Can you work these out from the model? Positions are in its coordinate system, mm. A direction names the side the tool comes from. Coordinates: 2 decimals unless noted, no trailing zeros. Loops run counter-clockwise (first coordinate to the right, second up) from the corner with the lowest first, then second, coordinate; pieces in that order, holes last. Notation, with made-up numbers: (64, 5) -> (83, 5) arc R18 ccw to (83, 14) -> close; hole circle Ø8 at (-15.5, -38). An arc over 180 degrees is marked (long way). Use one line per item in the form item = value. Start each with the question number.
(1) I'm going to push flat-ended pins straight in: pin 1 (2.5 mm diameter, centred on y = 11.5, z = 9.5, fed in from +X); pin 2 (3.5 mm diameter, centred on y = 4.45, z = 4, fed in from +X); pin 3 (2 mm diameter, centred on x = 5, z = 5, fed in from +Y); pin 4 (1 mm diameter, centred on y = 1.5, z = 13.5, fed in from +X). Where does each tip first touch, or does it pass through?
(2) Imagine slicing it at C-C (y = 4.45). List the corners of the cut face in (x, z) for me, plus the area to 3 significant figures.
(3) On a 3-axis mill with a long thin cutter (end or side, diameter ignored), from which of +Z, -Z, +X, -X, +Y, -Y can I reach the whole of each face in a straight line? I mean faces 4 (the flat face through (3, 7, 20)), 5 (the flat face through (5, 2, 10)), 6 (the cylindrical face through (1.97, 1.97, 12.21)), 7 (the flat face through (6.5, 7, 10)), 8 (the flat face through (5, 9.9, 10)). Say none if no direction works.
(4) Imagine slicing it at D-D (z = 4). List the corners of the cut face in (x, y) for me.
(5) Imagine slicing it at B-B (x = 1). List the corners of the cut face in (y, z) for me.
(6) Thinking about a two-plate mould opening in Y: for faces 1 (the flat face through (5.8, 4.3, 7.2)), 2 (the cylindrical face through (4.99, 5.66, 9.63)), 3 (the flat face through (3, 7, 0)), which applies, released by +Y, released by -Y, zero draft, split by the parting line, or undercut?
(7) I need wall thicknesses on line 1 (Y direction, x = 4.5, z = 10); line 2 (Y direction, x = 4.5, z = 4); line 3 (Z direction, x = 2, y = 4.45). Which ranges of each line are inside material? Lowest first, please. Write a range as [from, to].
(8) Imagine slicing it at A-A (z = 10). List the corners of the cut face in (x, y) for me, plus the area to 3 significant figures.
```python
from build123d import *

# Parameters (mm, degrees)
BOSS_EXTRUDE1_DEPTH                                  = 20
CUT_EXTRUDE1_DEPTH                                   = 20
HOLE_SIZE_PER_SOCKET_HEAD_CAP_SCREW_TYPE_D           = 3.4
HOLE_SIZE_PER_SOCKET_HEAD_CAP_SCREW_TYPE_DEPTH       = 10
HOLE_SIZE_PER_SOCKET_HEAD_CAP_SCREW_TYPE_CBORE_D     = 6
HOLE_SIZE_PER_SOCKET_HEAD_CAP_SCREW_TYPE_CBORE_DEPTH = 4
HOLE_SIZE_PER_SOCKET_HEAD_CAP_SCREW_TYPE_TIP         = 1.021463052
CHAMFER1_SIZE                                        = 1
SKETCH8_R                                            = 2
CUT_EXTRUDE2_DEPTH                                   = 8


with BuildPart() as part:
    # Sketch1 → Boss-Extrude1 (new body)
    with BuildSketch(Plane.XY):
        with BuildLine():
            Line((0, 0), (0, 13))
            Line((0, 13), (3.4, 13))
            Line((3.4, 13), (3.4, 10.558257569))
            ThreePointArc((3.4, 10.558257569), (3.246446609, 9.746446609), (4.058257569, 9.9))
            Line((4.058257569, 9.9), (6.5, 9.9))
            Line((6.5, 9.9), (6.5, 0))
            Line((6.5, 0), (0, 0))
        make_face()
    extrude(amount=BOSS_EXTRUDE1_DEPTH)

    # Sketch7 → Cut-Extrude1 (cut)
    with BuildSketch(Plane.XY.offset(20)):
        Polygon((6.5, 5), (5, 3.5), (5, 0), (6.5, 0), align=None)
    extrude(amount=-CUT_EXTRUDE1_DEPTH, mode=Mode.SUBTRACT)

    # Hole size per socket head cap screw type 0
    with Locations(Plane(origin=(0, 0, 0), x_dir=(0, 0, -1), z_dir=(-1, 0, 0))):
        with Locations((-10, -4)):
            CounterBoreHole(HOLE_SIZE_PER_SOCKET_HEAD_CAP_SCREW_TYPE_D / 2, HOLE_SIZE_PER_SOCKET_HEAD_CAP_SCREW_TYPE_CBORE_D / 2, HOLE_SIZE_PER_SOCKET_HEAD_CAP_SCREW_TYPE_CBORE_DEPTH, depth=HOLE_SIZE_PER_SOCKET_HEAD_CAP_SCREW_TYPE_DEPTH)
            with Locations((0, 0, -(HOLE_SIZE_PER_SOCKET_HEAD_CAP_SCREW_TYPE_DEPTH + HOLE_SIZE_PER_SOCKET_HEAD_CAP_SCREW_TYPE_TIP / 2))):  # 118° drill point
                Cone(0, HOLE_SIZE_PER_SOCKET_HEAD_CAP_SCREW_TYPE_D / 2, HOLE_SIZE_PER_SOCKET_HEAD_CAP_SCREW_TYPE_TIP, mode=Mode.SUBTRACT)

    # Chamfer1
    chamfer1_edges = [part.edges().sort_by_distance(p)[0] for p in [
        (2.5, 0, 20),
        (2.5, 0, 0),
    ]]
    chamfer(chamfer1_edges, length=CHAMFER1_SIZE)

    # Sketch8 → Cut-Extrude2 (cut)
    with BuildSketch(Plane.ZY):
        with Locations((4, 4.45)):
            Circle(SKETCH8_R)
    extrude(amount=-CUT_EXTRUDE2_DEPTH, mode=Mode.SUBTRACT)


solid = part.part
```
Worked out:
q1.pin_1 = 3.4
q1.pin_2 = through
q1.pin_3 = 9.9
q1.pin_4 = 5
q2.outline = (0, 0) -> (5.95, 0) -> (5.95, 2) -> (0, 2) -> close; (0, 6) -> (5.95, 6) -> (5.95, 8.36) -> (4, 8.36) -> (4, 7.03) -> (0, 7.03) -> close; (0, 12.97) -> (4, 12.97) -> (4, 11.64) -> (5.95, 11.64) -> (5.95, 20) -> (0, 20) -> close
q2.area = 65.1 mm2
q3.face_4 = +Z, +X, -X, +Y, -Y
q3.face_5 = +Z, -Z, +X, -Y
q3.face_6 = -X
q3.face_7 = +Z, -Z, +X, +Y, -Y
q3.face_8 = +Z, -Z, +X, +Y
q4.outline = (0, 0) -> (5, 0) -> (5, 2.45) -> (0, 2.45) -> close; (0, 6.45) -> (6.5, 6.45) -> (6.5, 9.9) -> (4.06, 9.9) arc R0.5 cw (long way) to (3.4, 10.56) -> (3.4, 13) -> (0, 13) -> close
q5.outline = (0, 1) -> (1, 0) -> (13, 0) -> (13, 20) -> (1, 20) -> (0, 19) -> close; hole circle Ø6 at (4, 10); hole circle Ø4 at (4.45, 4)
q6.face_1 = released by -Y
q6.face_2 = undercut
q6.face_3 = zero draft
q7.line_1 = [0, 2.3], [5.7, 9.9]
q7.line_2 = [0, 2.45], [6.45, 9.9]
q7.line_3 = [0, 2], [6, 7.03], [12.97, 20]
q8.outline = (0, 0) -> (5, 0) -> (5, 2.3) -> (4, 2.3) -> (4, 1) -> (0, 1) -> close; (0, 7) -> (4, 7) -> (4, 5.7) -> (6.5, 5.7) -> (6.5, 9.9) -> (4.06, 9.9) arc R0.5 cw (long way) to (3.4, 10.56) -> (3.4, 13) -> (0, 13) -> close
q8.area = 38.6 mm2
